Here's the drawing with two shaded views (mm, measured from the low corner). I have some questions. A direction names the side the tool comes from. Give positions to 0.01 mm unless a question says otherwise; leave off trailing zeros. Loops run counter-clockwise (first coordinate to the right, second up) from the corner with the lowest first, then second, coordinate; pieces in that order, holes last. Notation, with made-up numbers: M 62,-3.5 L 100,-3.5 A16 ccw 100,7.5 Z; hole C 89,-26 d1. An arc over 180 degrees is marked long. Use CSV: the item, a comma, the result in double quotes.
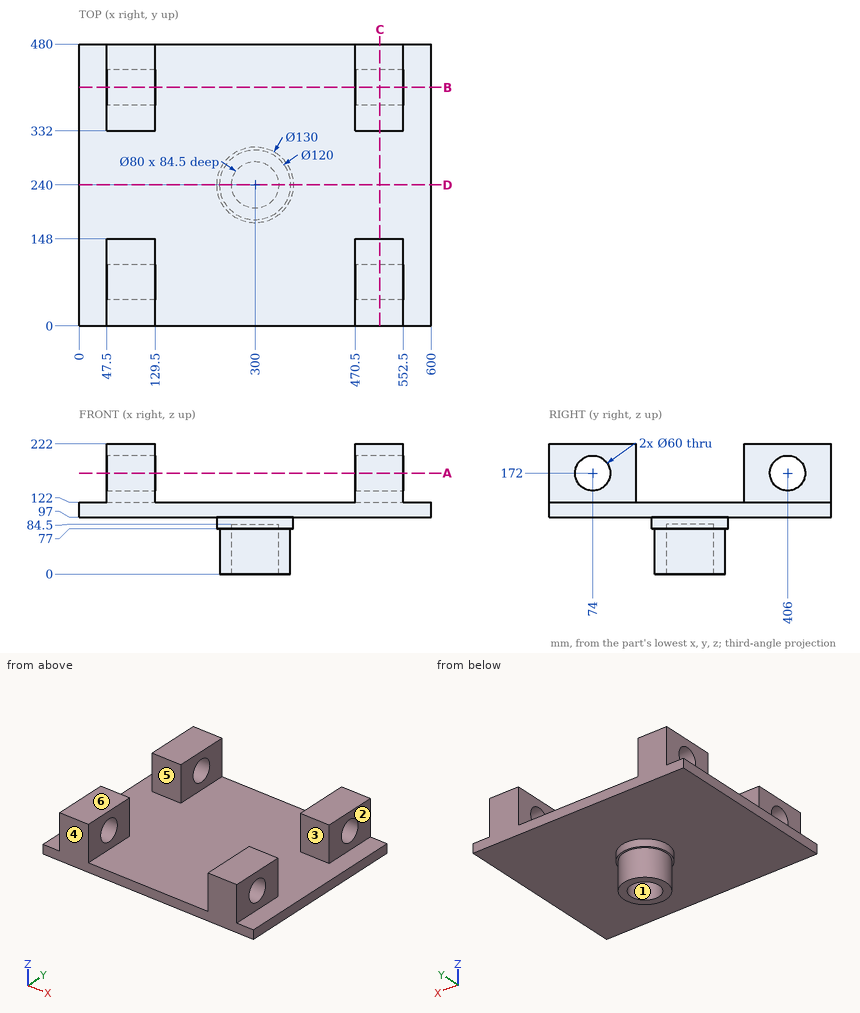
1. Please list where these lines run through material, in increasing order: line 1 (Y direction, x = 85, z = 172); line 2 (Z direction, x = 86.5, y = 74); line 3 (X direction, y = 27.5, z = 128.5).
Outcome:
line 1,"0 to 44, 104 to 148, 332 to 376, 436 to 480"
line 2,"97 to 142, 202 to 222"
line 3,"47.5 to 129.5, 470.5 to 552.5"
2. I want a section at A-A, the plane z = 172. Give the number of separate pieces and of enclosed holes in the cut face, then the cut area to 3 significant figures.
Outcome:
separate pieces,"8"
enclosed holes,"0"
area,"28,900 mm2"
3. I want a section at B-B, the plane y = 406. List the corners of the cut face in (x, z) for me, then the cut area to 3 significant figures.
Outcome:
outline,"M 0,97 L 600,97 L 600,122 L 552.5,122 L 552.5,142 L 470.5,142 L 470.5,122 L 129.5,122 L 129.5,142 L 47.5,142 L 47.5,122 L 0,122 Z; M 47.5,202 L 129.5,202 L 129.5,222 L 47.5,222 Z; M 470.5,202 L 552.5,202 L 552.5,222 L 470.5,222 Z"
area,"21,600 mm2"
4. I want a section at C-C, the plane x = 512.5. List the corners of the cut face in (y, z) for me.
Outcome:
outline,"M 0,97 L 480,97 L 480,222 L 332,222 L 332,122 L 148,122 L 148,222 L 0,222 Z; hole C 74,172 d60; hole C 406,172 d60"
5. Which directions (+Z, -Z, +X, -X, +Y, -Y) give clear straight access to the entire face, cutting with the end or side of a thin tool? Please do the marked faces 1, 2 and 3.
Outcome:
face 1,"-Z"
face 2,"+Z, +X, +Y, -Y"
face 3,"+Z, +X, -X"
6. If we mould it in two halves opening along Y, with no side actions, what happens to the marked faces 4, 5 and 6? For each: +Y half, -Y half, draft (parallel to the pull), parting line (faces both ways), or undercut.
Outcome:
face 4,"-Y half"
face 5,"undercut"
face 6,"draft"
7. I'm going to push flat-ended pins straight in: pin 1 Ø12 at (x, y) = (428, 50) entering from -Z; pin 2 Ø24 at (x, y) = (318, 236) entering from -Z. Where does each tip first touch, or does it pass through?
Outcome:
pin 1,"z = 97"
pin 2,"z = 84.5"
8. I want a section at D-D, the plane y = 240. List the corners of the cut face in (x, z) for me.
Outcome:
outline,"M 0,97 L 235,97 L 235,77 L 240,77 L 240,0 L 260,0 L 260,84.5 L 340,84.5 L 340,0 L 360,0 L 360,77 L 365,77 L 365,97 L 600,97 L 600,122 L 0,122 Z"
